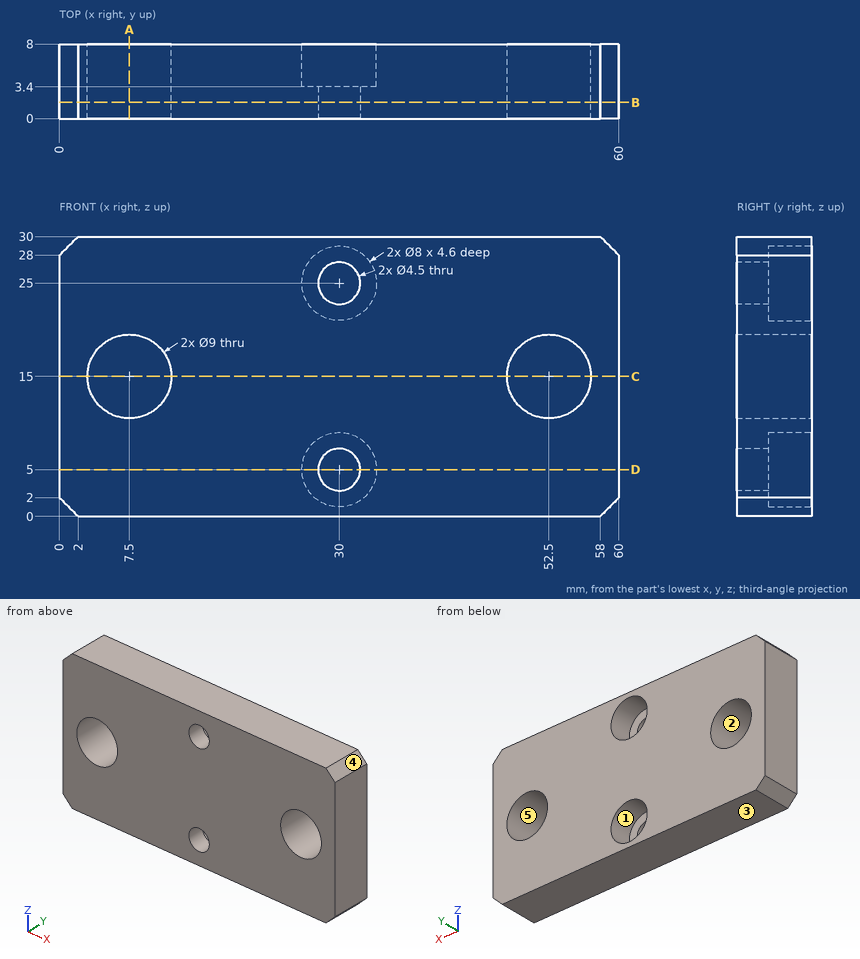
Source: three-view drawing plus pictorial views. Frame: mm from the lowest corner of the part. A direction names the side the tool comes from. Coordinates: 2 decimals unless noted, no trailing zeros. Loops run counter-clockwise (first coordinate to the right, second up) from the corner with the lowest first, then second, coordinate; pieces in that order, holes last. Notation, with made-up numbers: (21.5, -12.5) -> (33.5, -12.5) arc R22 ccw to (33.5, 22.5) -> close; hole circle Ø4 at (12.25, -0.5). An arc over 180 degrees is marked (long way). Answer in a Markdown table with one row per item. Add a question column.
Q1. Contact query for a flat-ended pin moving along its axis: pin 1 Ø5 at (x, z) = (30, 5) entering from +Y. Output: stop coordinate, or through.
Q2. Section B-B on y = 1.75. Return the cut outline in (x, z), and give its area (3 significant figures).
Q3. Pull-direction query (X, two-part tool) for the marked faces 3, 4 and 5; classes: pulls with the +X half, pulls with the -X half, needs draft (parallel to the pull), parting line crosses it, or undercut.
Q4. Section C-C on z = 15. Return the cut outline in (x, y).
Q5. Section D-D on z = 5. Return the cut outline in (x, y), and give its area (3 significant figures).
Q6. Reachability of the marked faces 1 and 2 from +Z, -Z, +X, -X, +Y, -Y: full face, straight path, thin tool, end or side. Return the list, or none.
Q7. Section A-A on x = 7.5. Return the cut outline in (y, z).
Q8. Ray query, line 1 along Z through (x, y) = (30, 6.8); line 2 along X through (y, z) = (4.75, 18); line 3 along Z through (x, y) = (30, 2.55). Return the intervals inside material, ascending.
Computed values:
| question | item | result |
|---|---|---|
| 1 | pin 1 | stops at y = 3.4 |
| 2 | outline | (0, 2) -> (2, 0) -> (58, 0) -> (60, 2) -> (60, 28) -> (58, 30) -> (2, 30) -> (0, 28) -> close; hole circle Ø9 at (7.5, 15); hole circle Ø4.5 at (30, 5); hole circle Ø4.5 at (30, 25); hole circle Ø9 at (52.5, 15) |
| 2 | area | 1,630 mm^2 |
| 3 | face 3 | needs draft |
| 3 | face 4 | pulls with the +X half |
| 3 | face 5 | undercut |
| 4 | outline | (0, 0) -> (3, 0) -> (3, 8) -> (0, 8) -> close; (12, 0) -> (48, 0) -> (48, 8) -> (12, 8) -> close; (57, 0) -> (60, 0) -> (60, 8) -> (57, 8) -> close |
| 5 | outline | (0, 0) -> (27.75, 0) -> (27.75, 3.4) -> (26, 3.4) -> (26, 8) -> (0, 8) -> close; (32.25, 0) -> (60, 0) -> (60, 8) -> (34, 8) -> (34, 3.4) -> (32.25, 3.4) -> close |
| 5 | area | 428 mm^2 |
| 6 | face 1 | +Y |
| 6 | face 2 | +Y, -Y |
| 7 | outline | (0, 0) -> (8, 0) -> (8, 10.5) -> (0, 10.5) -> close; (0, 19.5) -> (8, 19.5) -> (8, 30) -> (0, 30) -> close |
| 8 | line 1 | z = 0 to 1, 9 to 21, 29 to 30 |
| 8 | line 2 | x = 0 to 4.15, 10.85 to 49.15, 55.85 to 60 |
| 8 | line 3 | z = 0 to 2.75, 7.25 to 22.75, 27.25 to 30 |
